Can you work these out from the model? Positions are in its coordinate system, mm. A direction names the side the tool comes from. Give positions to 0.01 mm unless a question says otherwise; leave off trailing zeros. Write each loop counter-clockwise with the first axis right and the second up, starting at its lowest first coordinate (ties: lowest second). Pieces come first, ordered by that corner, then holes.
from build123d import *

# Parameters (mm, degrees)
SKETCH_1_R      = 270
EXTRUDE_1_DEPTH = 2


with BuildPart() as part:
    # 草图1 → 凸台-拉伸1 (new body)
    with BuildSketch(Plane.XY):
        Circle(SKETCH_1_R)
        Polygon((33.25966317, 13.776603565), (13.776603565, 33.25966317), (-13.776603565, 33.25966317), (-33.25966317, 13.776603565), (-33.25966317, -13.776603565), (-13.776603565, -33.25966317), (13.776603565, -33.25966317), (33.25966317, -13.776603565), align=None, mode=Mode.SUBTRACT)
    extrude(amount=EXTRUDE_1_DEPTH)


solid = part.part
(1) Will these pins go through, and if not, where does the flat tip stop? P1, Ø5, axis at x = 202, y = -152.5, coming from the -Z side; P2, Ø0.6, axis at x = -5, z = 1, coming from the +Y side.
Returned:
P1: stops at z = 0
P2: stops at y = 269.96
(2) If we mould it in two halves opening along Y, with no side actions, what happens to faces 1 (the face through (-4, -56, 0)), 2 (the face through (-23.382, 23.655, 0.986)), 3 (the face through (-214.263, -164.291, 0.986))? For each: +Y half, -Y half, draft (parallel to the pull), parting line (faces both ways), or undercut.
Returned:
face 1: draft
face 2: undercut
face 3: parting line
(3) If I drill on L1, parallel to X at y = 3, z = 1.2; L2, parallel to X at y = -7, z = 1.65; L3, parallel to Y at x = -64, z = 0.45, over which ranges is the centre line in solid material (lowest first)?
Returned:
L1: x = -269.98 to -33.26, 33.26 to 269.98
L2: x = -269.91 to -33.26, 33.26 to 269.91
L3: y = -262.31 to 262.31
(4) For faces 4 (the face through (23.382, -23.655, 0.986)), 5 (the face through (-4, -56, 2)), which set-ups out of +Z, -Z, +X, -X, +Y, -Y let a thin tool reach every point of the face, with its end or its side?
Returned:
face 4: +Z, -Z
face 5: +Z, +X, -X, +Y, -Y
(5) Imagine slicing it at D-D, the plane y = 150.5. Write out the boundary of the cut face in (x, z).
Returned:
outline: (-224.16, 0) - (224.16, 0) - (224.16, 2) - (-224.16, 2) - close
(6) Imagine slicing it at A-A, the plane x = 0. Write out the boundary of the cut face in (y, z).
Returned:
outline: (-270, 0) - (-33.26, 0) - (-33.26, 2) - (-270, 2) - close; (33.26, 0) - (270, 0) - (270, 2) - (33.26, 2) - close
(7) Imagine slicing it at B-B, the plane z = 1.55. Write out the boundary of the cut face in (x, y).
Returned:
outline: circle Ø540 at (0, 0); hole (-33.26, -13.78) - (-13.78, -33.26) - (13.78, -33.26) - (33.26, -13.78) - (33.26, 13.78) - (13.78, 33.26) - (-13.78, 33.26) - (-33.26, 13.78) - close
